Read the model definition and answer for the solid it produces. Units are mm, in the model's axes. A direction names the side the tool comes from. Give positions to 0.01 mm unless a question says otherwise; leave off trailing zeros. Loops run counter-clockwise (first coordinate to the right, second up) from the corner with the lowest first, then second, coordinate; pieces in that order, holes last. Notation, with made-up numbers: (-38.75, 39) - (18.25, 39) arc R23 ccw to (18.25, 50) - close; hole circle Ø1 at (25.5, 30.25). An arc over 180 degrees is marked (long way). Write item = value, one per line.
```python
from build123d import *

# Parameters (mm, degrees)
SKETCH1_R           = 0.95
BOSS_EXTRUDE1_DEPTH = 1.3


with BuildPart() as part:
    # Sketch1 → Boss-Extrude1 (new body)
    with BuildSketch(Plane.XY):
        with BuildLine():
            ThreePointArc((-6.005563392, -9.696368719), (-4.019375294, -9.84339787), (-3.384498187, -11.731119191))
            Line((-3.384498187, -11.731119191), (-4.128163769, -14.506516929))
            ThreePointArc((-4.128163769, -14.506516929), (0, 16.85), (4.128163769, -14.506516929))
            Line((4.128163769, -14.506516929), (3.384498187, -11.731119191))
            ThreePointArc((3.384498187, -11.731119191), (4.019375294, -9.84339787), (6.005563392, -9.696368719))
            ThreePointArc((6.005563392, -9.696368719), (8.494705662, -10.109304713), (10.669798447, -8.830509674))
            ThreePointArc((10.669798447, -8.830509674), (0, 13.85), (-10.669798447, -8.830509674))
            ThreePointArc((-10.669798447, -8.830509674), (-8.494705662, -10.109304713), (-6.005563392, -9.696368719))
        make_face()
        with Locations((5.123164674, -11.26524491)):
            Circle(SKETCH1_R, mode=Mode.SUBTRACT)
        with Locations((-5.123164674, -11.26524491)):
            Circle(SKETCH1_R, mode=Mode.SUBTRACT)
    extrude(amount=BOSS_EXTRUDE1_DEPTH)


solid = part.part
```
1) This flat-tipped pin is pushed along its axis until it touches: P1, Ø1.5, axis at x = -5.12, y = -11.27, coming from the -Z side. Where does it stop, or does it pass through?
Output:
P1 = through
2) Find the intervals of material crossed by probe 1 along X at (y, z) = (-12, 0.1); probe 2 along X at (y, z) = (-5.5, 1.2); probe 3 along X at (y, z) = (9, 0.4), in increasing order.
Output:
probe_1 = -9.38 to -5.73, -4.52 to -3.46, 3.46 to 4.52, 5.73 to 9.38
probe_2 = -14.61 to -12.71, 12.71 to 14.61
probe_3 = -13.74 to -10.53, 10.53 to 13.74
3) A tool of negligible diameter and unlimited length cuts with its end or side. For faces 1 (the face through (0, 14, 1.3)), 2 (the face through (-3.75, -13.1, 0.64)), 3 (the face through (-8.53, -10.103, 0.641)), from which of +Z, -Z, +X, -X, +Y, -Y can it reach the whole face along a straight path? Write none if from no direction.
Output:
face_1 = +Z, +X, -X, +Y, -Y
face_2 = +Z, -Z, -Y
face_3 = +Z, -Z
4) The mould has two halves that part along X. Classify faces 4 (the face through (0, 14, 0)), 5 (the face through (-0.643, 16.837, 0.641)), 6 (the face through (4, -9.86, 0.64)), 7 (the face through (0.439, 13.843, 0.641)): pulls with the +X half, pulls with the -X half, needs draft (parallel to the pull), parting line crosses it, or undercut.
Output:
face_4 = needs draft
face_5 = parting line crosses it
face_6 = undercut
face_7 = undercut
5) A cutting plane is placed at D-D on x = 0. Determine the outline of the cut face in (y, z).
Output:
outline = (13.85, 0) - (16.85, 0) - (16.85, 1.3) - (13.85, 1.3) - close
6) A cutting plane is placed at B-B on x = -6.5. Determine the outline of the cut face in (y, z), then the cut area to 3 significant figures.
Output:
outline = (-13.67, 0) - (-9.93, 0) - (-9.93, 1.3) - (-13.67, 1.3) - close; (12.23, 0) - (15.47, 0) - (15.47, 1.3) - (12.23, 1.3) - close
area = 9.06 mm²
7) A cutting plane is placed at C-C on z = 0.45. Determine the outline of the cut face in (x, y).
Output:
outline = (-10.67, -8.83) arc R13.85 cw (long way) to (10.67, -8.83) arc R3.7 cw to (6.01, -9.7) arc R1.8 ccw to (3.38, -11.73) - (4.13, -14.51) arc R15.95 ccw (long way) to (-4.13, -14.51) - (-3.38, -11.73) arc R1.8 ccw to (-6.01, -9.7) arc R3.7 cw to start; hole circle Ø1.9 at (-5.12, -11.27); hole circle Ø1.9 at (5.12, -11.27)
8) A cutting plane is placed at A-A on y = -7.5. Determine the outline of the cut face in (x, z).
Output:
outline = (-13.56, 0) - (-11.64, 0) - (-11.64, 1.3) - (-13.56, 1.3) - close; (11.64, 0) - (13.56, 0) - (13.56, 1.3) - (11.64, 1.3) - close
